```python
from build123d import *

# Parameters (mm, degrees)
RAIL_BODY_580_DEPTH        = 580
MOUNTING_HOLES_SKETCH_R    = 5
MOUNTING_HOLES_5X_10_DEPTH = 580


with BuildPart() as part:
    # Rail Profile Sketch → Rail Body 580 (new body)
    with BuildSketch(Plane(origin=(0, 0, 0), x_dir=(0, 0, -1), z_dir=(1, 0, 0))):
        with BuildLine():
            Line((-30, 10), (-30, 23))
            ThreePointArc((-30, 23), (-28.535533906, 26.535533906), (-25, 28))
            Line((-25, 28), (30, 28))
            Line((30, 28), (30, 0))
            Line((30, 0), (15, 0))
            Line((15, 0), (15, 8))
            Line((15, 8), (-1, 8))
            Line((-1, 8), (-1, 0))
            Line((-1, 0), (-20, 0))
            Line((-20, 0), (-30, 10))
        make_face()
    extrude(amount=RAIL_BODY_580_DEPTH)

    # Mounting Holes Sketch → Mounting Holes 5xØ10 (cut)
    with BuildSketch(Plane(origin=(0, 28, 0), x_dir=(1, 0, 0), z_dir=(0, 1, 0))):
        with Locations(Location((25, 7, 0), (0, 0, 270))):
            Circle(MOUNTING_HOLES_SKETCH_R)
        with Locations(Location((157.5, 7, 0), (0, 0, 270))):
            Circle(MOUNTING_HOLES_SKETCH_R)
        with Locations(Location((290, 7, 0), (0, 0, 270))):
            Circle(MOUNTING_HOLES_SKETCH_R)
        with Locations(Location((422.5, 7, 0), (0, 0, 270))):
            Circle(MOUNTING_HOLES_SKETCH_R)
        with Locations(Location((555, 7, 0), (0, 0, 270))):
            Circle(MOUNTING_HOLES_SKETCH_R)
    extrude(amount=-MOUNTING_HOLES_5X_10_DEPTH, mode=Mode.SUBTRACT)


solid = part.part
```
Geometry: final body of the model. Coordinates: model frame, mm. A direction names the side the tool comes from. Coordinates: 2 decimals unless noted, no trailing zeros. Order: outer loops, then holes, each group sorted by start corner. A loop starts at its lowest first (then second) coordinate and runs counter-clockwise, first axis right, second up. Notation, with made-up numbers: (72, 82) - (84, 82) arc R23 ccw to (84, 100) - close; hole circle Ø10 at (39, 1.25). An arc over 180 degrees is marked (long way). Return JSON: item names as keys, results as strings. Group by question number.
1. Set-up query: faces 4 (the face through (286, 8, -11)), 5 (the face through (286, 0, -23)). Return all of +Z, -Z, +X, -X, +Y, -Y with unobstructed straight access to the full face (end or side cutting, diameter ignored); none if empty.
2. Pin query (flat end, axial travel): pin 1 (13 mm diameter, centred on x = 555, z = -7, fed in from -Y); pin 2 (6 mm diameter, centred on x = 290, z = -7, fed in from -Y); pin 3 (6 mm diameter, centred on x = 206, y = 4.5, fed in from +Z); pin 4 (6.5 mm diameter, centred on x = 349, y = 5.5, fed in from +Z). Return the tip coordinate at first contact, or that it passes through.
3. Cut plane B-B (x = 290). Output: boundary loops of the cut face in (y, z), plus the area to 3 significant figures.
4. Pull-direction query (X, two-part tool) for faces 1 (the face through (0, 14, 0)), 2 (the face through (20.564, 18.14, -4.693)), 3 (the face through (286, 5, 25)); classes: pulls with the +X half, pulls with the -X half, needs draft (parallel to the pull), parting line crosses it, or undercut.
5. Cut plane A-A (z = -7). Output: boundary loops of the cut face in (x, y).
6. Material intervals for line 1 along X through (y, z) = (18.5, -7); line 2 along X through (y, z) = (21.25, -6); line 3 along Z through (x, y) = (422.5, 20.5), sorted ascending. Write a range as [from, to].
7. Cut plane C-C (x = 452.5). Output: boundary loops of the cut face in (y, z).
Resolved:
{
 "1": {"face 4": "+X, -X, -Y", "face 5": "+Z, -Z, +X, -X, -Y"},
 "2": {"pin 1": "stops at y = 8", "pin 2": "passes through", "pin 3": "stops at z = 27.5", "pin 4": "stops at z = 28.75"},
 "3": {"outline": "(0, -30) - (28, -30) - (28, -12) - (8, -12) - (8, -15) - (0, -15) - close; (0, 1) - (8, 1) - (8, -2) - (28, -2) - (28, 25) arc R5 ccw to (23, 30) - (10, 30) - (0, 20) - close", "area": "1,300 mm²"},
 "4": {"face 1": "pulls with the -X half", "face 2": "undercut", "face 3": "needs draft"},
 "5": {"outline": "(0, 8) - (20, 8) - (20, 28) - (0, 28) - close; (30, 8) - (152.5, 8) - (152.5, 28) - (30, 28) - close; (162.5, 8) - (285, 8) - (285, 28) - (162.5, 28) - close; (295, 8) - (417.5, 8) - (417.5, 28) - (295, 28) - close; (427.5, 8) - (550, 8) - (550, 28) - (427.5, 28) - close; (560, 8) - (580, 8) - (580, 28) - (560, 28) - close"},
 "6": {"line 1": "x = [0, 20], [30, 152.5], [162.5, 285], [295, 417.5], [427.5, 550], [560, 580]", "line 2": "x = [0, 20.1], [29.9, 152.6], [162.4, 285.1], [294.9, 417.6], [427.4, 550.1], [559.9, 580]", "line 3": "z = [-30, -12], [-2, 30]"},
 "7": {"outline": "(0, -30) - (28, -30) - (28, 25) arc R5 ccw to (23, 30) - (10, 30) - (0, 20) - (0, 1) - (8, 1) - (8, -15) - (0, -15) - close"}
}
